```python
from build123d import *

# Parameters (mm, degrees)
FILLET1_R          = 0.25
FILLET2_R          = 1.8
SKETCH5_W          = 12
SKETCH5_H          = 1.6
CUT_EXTRUDE1_DEPTH = 1.4


with BuildPart() as part:
    # Sketch2 → Base-Revolve (revolve)
    with BuildSketch(Plane.XY, mode=Mode.PRIVATE) as base_revolve_sk:
        Polygon((0, 0), (19.6, 0), (19.6, 3), (5.6, 3), (5.198, 2.598), (3.6, 2.598), (3.6, 6), (0, 5.685040811), align=None)
    revolve(base_revolve_sk.sketch.rotate(Axis((-3.442001378, 0, 0), (1, 0, 0)), 90), axis=Axis((-3.442001378, 0, 0), (1, 0, 0)))

    # Fillet1
    fillet1_edges = [part.edges().sort_by_distance(p)[0] for p in [
        (3.6, 0, -2.598),
        (5.198, 0, -2.598),
    ]]
    fillet(fillet1_edges, radius=FILLET1_R)

    # Fillet2
    fillet2_edges = [part.edges().sort_by_distance(p)[0] for p in [
        (0, 0, -5.685040811),
    ]]
    fillet(fillet2_edges, radius=FILLET2_R)

    # Sketch5 → Cut-Extrude1 (cut)
    with BuildSketch(Plane(origin=(0, 0, 0), x_dir=(0, 0, -1), z_dir=(1, 0, 0))):
        Rectangle(SKETCH5_W, SKETCH5_H)
    extrude(amount=CUT_EXTRUDE1_DEPTH, mode=Mode.SUBTRACT)

    # Sketch3 → Cut-Revolve1 (revolve, cut)
    with BuildSketch(Plane.XY, mode=Mode.PRIVATE) as cut_revolve1_sk:
        Polygon((19.105416006, 3), (20.105416006, 3), (19.6, 2.134), align=None)
    revolve(cut_revolve1_sk.sketch.rotate(Axis((-0.122578865, 0, 0), (1, 0, 0)), 90), axis=Axis((-0.122578865, 0, 0), (1, 0, 0)), mode=Mode.SUBTRACT)


solid = part.part
```
The listing builds one solid part. Answer for the finished solid, in the listing's coordinates (mm). A direction names the side the tool comes from. Give positions to 0.01 mm unless a question says otherwise; leave off trailing zeros. Write each loop counter-clockwise with the first axis right and the second up, starting at its lowest first coordinate (ties: lowest second). Pieces come first, ordered by that corner, then holes. Notation, with made-up numbers: (38, -32.5) - (94, -32.5) arc R18 cw to (94, -23.5) - close; hole circle Ø7 at (49, -9). An arc over 180 degrees is marked (long way). Use one line per item in the form item = value. Start each with the question number.
1) Consider line 1 along X through (y, z) = (3.5, 2.25); line 2 along Y through (x, z) = (18.25, -1.5); line 3 along Y through (x, z) = (8.25, 0). Determine where each line is inside the solid, lowest interval first. Write a range as from..to.
2) Flat-ended cylindrical pins translate along their axes: pin 1 Ø0.7 at (x, z) = (0.5, 0.5) entering from -Y; pin 2 Ø1 at (y, z) = (-3, -4.5) entering from -X; pin 3 Ø5 at (x, y) = (8.5, 0.5) entering from +Z; pin 4 Ø3 at (x, z) = (3.5, 1.5) entering from -Y. Find the tip coordinate at first contact, or state that the pin passes through.
3) The mould has two halves that part along X. Classify faces 1 (the face through (0, -2, 0)), 2 (the face through (4.464, 2.305, 1.199)), 3 (the face through (19.6, 0, 0)), 4 (the face through (12.26, -0.9, 2.86)): pulls with the +X half, pulls with the -X half, needs draft (parallel to the pull), parting line crosses it, or undercut.
4) Find section A-A on x = 8. Determine the outline of the cut face in (y, z).
5) Find section B-B on x = 4.75. Determine the outline of the cut face in (y, z).
6) A tool of negligible diameter and unlimited length cuts with its end or side. For faces 5 (the face through (1, 0.8, 0)), 6 (the face through (2.173, -5.825, -0.765)), from which of +Z, -Z, +X, -X, +Y, -Y can it reach the whole face along a straight path? Write none if from no direction.
Geometry results:
q1.line_1 = 0..3.6
q1.line_2 = -2.6..2.6
q1.line_3 = -3..3
q2.pin_1 = -5.54
q2.pin_2 = 0.23
q2.pin_3 = 3
q2.pin_4 = -6
q3.face_1 = pulls with the -X half
q3.face_2 = undercut
q3.face_3 = pulls with the +X half
q3.face_4 = needs draft
q4.outline = circle Ø6 at (0, 0)
q5.outline = circle Ø5.2 at (0, 0)
q6.face_5 = +Z, -Z, -X
q6.face_6 = -X
